```python
from build123d import *

# Parameters (mm, degrees)
SKETCH1_R      = 2.4585
BASENUT_DEPTH  = 3.92
EXTRUDE1_START = 4.08
SKETCH2_R      = 4.89
SKETCH2_R_2    = 2.4585
EXTRUDE1_DEPTH = 4.08
CHAMFER1_SIZE  = 0.1956


with BuildPart() as part:
    # Sketch1 → BaseNut (new body)
    with BuildSketch(Plane.XY):
        Polygon((2.886751346, -5), (5.773502692, 0), (2.886751346, 5), (-2.886751346, 5), (-5.773502692, 0), (-2.886751346, -5), align=None)
        Circle(SKETCH1_R, mode=Mode.SUBTRACT)
    extrude(amount=-BASENUT_DEPTH)

    # Sketch3 → Double-Chamfer (revolve, cut)
    with BuildSketch(Plane(origin=(0, 0, 0), x_dir=(1, 0, 0), z_dir=(0, 1, 0)), mode=Mode.PRIVATE) as double_chamfer_sk:
        Polygon((4.44, 3.92), (5.773502692, 3.92), (5.773502692, 3.150101862), align=None)
        Polygon((5.773502692, 0.769898138), (4.44, 0), (5.773502692, 0), align=None)
    revolve(double_chamfer_sk.sketch.rotate(Axis((0, 0, -16.31077227), (0, 0, 1)), 179.999999973), axis=Axis((0, 0, -16.31077227), (0, 0, 1)), mode=Mode.SUBTRACT)

    # Sketch2 → Extrude1 (add)
    with BuildSketch(Plane(origin=(20.087129569, -4.281493882, 0), x_dir=(1, 0, 0), z_dir=(0, 0, 1)).offset(EXTRUDE1_START)):
        with Locations((-20.087129569, 4.281493882)):
            Circle(SKETCH2_R)
        with Locations((-20.087129569, 4.281493882)):
            Circle(SKETCH2_R_2, mode=Mode.SUBTRACT)
    extrude(amount=-EXTRUDE1_DEPTH)

    # Sketch5 → EndChamfer (revolve, cut)
    with BuildSketch(Plane(origin=(0, 0, 0), x_dir=(1, 0, 0), z_dir=(0, 1, 0))):
        Polygon((2.4585, 3.92), (3.375, 3.92), (2.4585, 3.0035), align=None)
    revolve(axis=Axis((0, 0, -16.800797033), (0, 0, 1)), mode=Mode.SUBTRACT)

    # Chamfer1
    chamfer1_edges = [part.edges().sort_by_distance(p)[0] for p in [
        (-4.89, 0, 4.08),
    ]]
    chamfer(chamfer1_edges, length=CHAMFER1_SIZE)


solid = part.part
```
The listing builds one solid part. Answer for the finished solid, in the listing's coordinates (mm). Coordinates: 2 decimals unless noted, no trailing zeros. Loops run counter-clockwise (first coordinate to the right, second up) from the corner with the lowest first, then second, coordinate; pieces in that order, holes last. Notation, with made-up numbers: M 38,72.25 L 51,72.25 A21 cw 51,89.25 Z; hole C -7,-13.5 d8. An arc over 180 degrees is marked long. Answer as CSV lines item,"result". Start each with the question number.
(1) The part is cut by section B-B (z = -1.5). Give the vertices of the cut face in (x, y), and give its area (3 significant figures).
(2) The part is cut by section C-C (z = 3.5). Give the vertices of the cut face in (x, y), and give its area (3 significant figures).
(3) Find the intervals of material crossed by L1, parallel to Y at x = 0, z = 1.25; L2, parallel to Z at x = 4.75, y = -0.5; L3, parallel to X at y = 1.5, z = -1.25, in increasing order. Write a range as [from, to].
(4) Given pin 1 (2 mm diameter, centred on y = -1.5, z = 0, fed in from -X); pin 2 (3 mm diameter, centred on y = -3, z = 2.5, fed in from +X), each flat-ended and moving along its own axis, determine where each tip first touches the part or whether it passes through.
(5) The mould has two halves that part along X. Classify faces 1 (the flat face through (4.35, 2.465, -1.937)), 2 (the flat face through (3, 2, -3.92)), 3 (the cylindrical face through (2.345, 0.738, 0.588)), 4 (the cylindrical face through (-1.06, -4.774, 1.969)): pulls with the +X half, pulls with the -X half, needs draft (parallel to the pull), parting line crosses it, or undercut.
Determined:
1,outline,"M -5.77,0 L -2.89,-5 L 2.89,-5 L 5.77,0 L 2.89,5 L -2.89,5 Z; hole C 0,0 d4.92"
1,area,"67.6 mm2"
2,outline,"C 0,0 d9.78; hole C 0,0 d4.92"
2,area,"56.1 mm2"
3,L1,"[-4.89, -2.46], [2.46, 4.89]"
3,L2,"[-3.73, -0.19], [0, 4]"
3,L3,"[-4.91, -1.95], [1.95, 4.91]"
4,pin 1,"x = -5.38"
4,pin 2,"x = 4.65"
5,face 1,"pulls with the +X half"
5,face 2,"needs draft"
5,face 3,"undercut"
5,face 4,"parting line crosses it"
